Build history of the part. All positions in model axes, mm. A direction names the side the tool comes from. Give positions to 0.01 mm unless a question says otherwise; leave off trailing zeros. Order: outer loops, then holes, each group sorted by start corner. A loop starts at its lowest first (then second) coordinate and runs counter-clockwise, first axis right, second up. Notation, with made-up numbers: (51, 76) - (109, 76) arc R28 cw to (109, 115) - close; hole circle Ø5 at (67.25, 54.25). An arc over 180 degrees is marked (long way). Write each question's results on one line, items separated by ' | '. Start each with the question number.
1) Cut at C-C on x = 35. List the corners of the cut face in (y, z).
2) Tool access for faces 5 (the face through (26.5, 1.5, 17.6)), 6 (the face through (-1.32, 11.66, 29.97)), 7 (the face through (18.765, 0.761, 31.117)): list every direction of +Z, -Z, +X, -X, +Y, -Y with a clear straight run to the whole face (end or side of a thin tool).
3) Two-plate mould, pull along Y, no slides. Class faces 1 (the face through (13, 23, -13)), 2 (the face through (-36.464, 0.761, -0.325)), 3 (the face through (-31.232, 12.346, 4.101)), 4 (the face through (-1, 25, -8)): +Y half, -Y half, draft (parallel to the pull), parting line (faces both ways), or undercut.
4) Drop flat-ended pins along their axis: pin 1 Ø3.5 at (x, z) = (-35, 0) entering from -Y; pin 2 Ø5 at (x, z) = (35, 0) entering from +Y; pin 3 Ø2.5 at (x, z) = (35, 0) entering from -Y; pin 4 Ø3 at (y, z) = (-19.5, 11) entering from +X. Give the stop position or say it passes through.
5) Drill centre lines: line 1 along X through (y, z) = (1.05, 0); line 2 along X through (y, z) = (14, 0); line 3 along Y through (x, z) = (26, -25.5). Where is each one in solid material? Low to high. Write a range as from..to.
6) Cut at B-B on z = 0. State how many separate pieces and enclosed holes the cut face has, plus the area to 3 significant figures.
7) Cut at A-A on y = 18. List the corners of the cut face in (x, z).
8) Cut at D-D on y = -7.5. List the corners of the cut face in (x, z), plus the area to 3 significant figures.
from build123d import *

# Parameters (mm, degrees)
SKETCH2_R           = 1.5
CUT_EXTRUDE1_DEPTH  = 62.846584384
SKETCH3_R           = 30
BOSS_EXTRUDE1_DEPTH = 2
SKETCH4_R           = 3.481990468
CUT_EXTRUDE2_DEPTH  = 2
SKETCH5_R           = 17.5
BOSS_EXTRUDE2_DEPTH = 35
SKETCH6_R           = 13
BOSS_EXTRUDE3_DEPTH = 15
FILLET1_R           = 12


with BuildPart() as part:
    # Sketch1 → Revolve1 (revolve)
    with BuildSketch(Plane.XY, mode=Mode.PRIVATE) as revolve1_sk:
        Polygon((-40, 0), (-30, 0), (-30, 25), (-40, 25), (-40, 23.5), (-31.5, 23.5), (-31.5, 1.5), (-40, 1.5), align=None)
    revolve(revolve1_sk.sketch.rotate(Axis((0, 0, 0), (0, 1, 0)), 270), axis=Axis((0, 0, 0), (0, 1, 0)))

    # Sketch2 → Cut-Extrude1 (cut, through all)
    with BuildSketch(Plane(origin=(0, 25, 0), x_dir=(1, 0, 0), z_dir=(0, 1, 0))):
        with Locations(Location((-35, 0, 0), (0, 0, 270))):
            Circle(SKETCH2_R)
        with Locations(Location((-17.5, 30.310889132, 0), (0, 0, 270))):
            Circle(SKETCH2_R)
        with Locations(Location((17.5, 30.310889132, 0), (0, 0, 270))):
            Circle(SKETCH2_R)
        with Locations(Location((35, 0, 0), (0, 0, 270))):
            Circle(SKETCH2_R)
        with Locations(Location((17.5, -30.310889132, 0), (0, 0, 270))):
            Circle(SKETCH2_R)
        with Locations(Location((-17.5, -30.310889132, 0), (0, 0, 270))):
            Circle(SKETCH2_R)
    extrude(amount=-CUT_EXTRUDE1_DEPTH, mode=Mode.SUBTRACT)

    # Sketch3 → Boss-Extrude1 (add)
    with BuildSketch(Plane(origin=(0, 25, 0), x_dir=(1, 0, 0), z_dir=(0, 1, 0))):
        with Locations(Location((0, 0, 0), (0, 0, 90))):
            Circle(SKETCH3_R)
    extrude(amount=-BOSS_EXTRUDE1_DEPTH)

    # Sketch4 → Cut-Extrude2 (cut)
    with BuildSketch(Plane(origin=(0, 23, 0), x_dir=(-1, 0, 0), z_dir=(0, -1, 0))):
        with Locations(Location((0, 0, 0), (0, 0, 90))):
            Circle(SKETCH4_R)
    extrude(amount=-CUT_EXTRUDE2_DEPTH, mode=Mode.SUBTRACT)

    # Sketch5 → Boss-Extrude2 (add)
    with BuildSketch(Plane(origin=(0, 23, 0), x_dir=(-1, 0, 0), z_dir=(0, -1, 0))):
        with Locations(Location((0, 0, 0), (0, 0, 270))):
            Circle(SKETCH5_R)
    extrude(amount=BOSS_EXTRUDE2_DEPTH)

    # Sketch6 → Boss-Extrude3 (add)
    with BuildSketch(Plane(origin=(0, -12, 0), x_dir=(-1, 0, 0), z_dir=(0, -1, 0))):
        with Locations(Location((0, 0, 0), (0, 0, 90))):
            Circle(SKETCH6_R)
    extrude(amount=BOSS_EXTRUDE3_DEPTH)

    # Fillet1
    fillet1_edges = [part.edges().sort_by_distance(p)[0] for p in [
        (0, -27, 13),
    ]]
    fillet(fillet1_edges, radius=FILLET1_R)


solid = part.part
Results:
1) outline: (0, -19.36) - (1.5, -19.36) - (1.5, -1.5) - (0, -1.5) - close; (0, 1.5) - (1.5, 1.5) - (1.5, 19.36) - (0, 19.36) - close; (23.5, -19.36) - (25, -19.36) - (25, -1.5) - (23.5, -1.5) - close; (23.5, 1.5) - (25, 1.5) - (25, 19.36) - (23.5, 19.36) - close
2) face 5: none | face 6: -Y | face 7: +Y, -Y
3) face 1: -Y half | face 2: draft | face 3: undercut | face 4: +Y half
4) pin 1: y = 0 | pin 2: y = 25 | pin 3: through | pin 4: x = 7.74
5) line 1: -40..-36.5, -33.5..-30, -17.5..17.5, 30..33.5, 36.5..40 | line 2: -31.5..-30, -17.5..17.5, 30..31.5 | line 3: 0..1.5, 23.5..25
6) separate pieces: 5 | enclosed holes: 0 | area: 1,770 mm^2
7) outline: circle Ø63 at (0, 0); circle Ø35 at (0, 0); hole circle Ø60 at (0, 0)
8) outline: circle Ø35 at (0, 0) | area: 962 mm^2
